The listing builds one solid part. Answer for the finished solid, in the listing's coordinates (mm). A direction names the side the tool comes from. Coordinates: 2 decimals unless noted, no trailing zeros. Write each loop counter-clockwise with the first axis right and the second up, starting at its lowest first coordinate (ties: lowest second). Pieces come first, ordered by that corner, then holes.
from build123d import *

# Parameters (mm, degrees)
SKETCH1_R           = 2.5
BOSS_EXTRUDE1_DEPTH = 10
SKETCH2_R           = 5
BOSS_EXTRUDE2_DEPTH = 10
SKETCH3_R           = 8
BOSS_EXTRUDE3_DEPTH = 10


with BuildPart() as part:
    # Sketch1 → Boss-Extrude1 (new body)
    with BuildSketch(Plane.XY):
        Circle(SKETCH1_R)
    extrude(amount=BOSS_EXTRUDE1_DEPTH)

    # Sketch2 → Boss-Extrude2 (add)
    with BuildSketch(Plane.XY.offset(10)):
        Circle(SKETCH2_R)
    extrude(amount=BOSS_EXTRUDE2_DEPTH)

    # Sketch3 → Boss-Extrude3 (add)
    with BuildSketch(Plane.XY.offset(20)):
        Circle(SKETCH3_R)
    extrude(amount=BOSS_EXTRUDE3_DEPTH)


solid = part.part
1. Flat-ended cylindrical pins translate along their axes: P1, Ø5, axis at x = -4, y = 3.5, coming from the -Z side; P2, Ø1, axis at x = -2, z = 13.5, coming from the +Y side; P3, Ø1, axis at x = -4.5, y = -6, coming from the -Z side. Find the tip coordinate at first contact, or state that the pin passes through.
Results found:
P1: stops at z = 10
P2: stops at y = 4.77
P3: stops at z = 20
2. Section C-C on z = 17 is taken. Give the vertices of the cut face in (x, y), then the cut area to 3 significant figures.
Results found:
outline: circle Ø10 at (0, 0)
area: 78.5 mm2
3. Section D-D on x = 3.5 is taken. Give the vertices of the cut face in (y, z), then the cut area to 3 significant figures.
Results found:
outline: (-7.19, 20) - (-3.57, 20) - (-3.57, 10) - (3.57, 10) - (3.57, 20) - (7.19, 20) - (7.19, 30) - (-7.19, 30) - close
area: 215 mm2
4. A tool of negligible diameter and unlimited length cuts with its end or side. For faces 1 (the cylindrical face through (-0.54, -2.44, 4.93)), 2 (the cylindrical face through (-1.73, -7.81, 24.93)), from which of +Z, -Z, +X, -X, +Y, -Y can it reach the whole face along a straight path? Write none if from no direction.
Results found:
face 1: -Z
face 2: +Z, -Z
5. Find the intervals of material crossed by L1, parallel to Z at x = -5, y = 5; L2, parallel to X at y = 1, z = 17.75; L3, parallel to X at y = 2, z = 5.25, in increasing order.
Results found:
L1: z = 20 to 30
L2: x = -4.9 to 4.9
L3: x = -1.5 to 1.5
6. Section A-A on x = 0 is taken. Give the vertices of the cut face in (y, z), then the cut area to 3 significant figures.
Results found:
outline: (-8, 20) - (-5, 20) - (-5, 10) - (-2.5, 10) - (-2.5, 0) - (2.5, 0) - (2.5, 10) - (5, 10) - (5, 20) - (8, 20) - (8, 30) - (-8, 30) - close
area: 310 mm2
